```python
from build123d import *

# Parameters (mm, degrees)
BASE_PLATE_10MM_DEPTH         = 10
SUPPORT_BLOCK_50MM_DEPTH      = 25
SUPPORT_BLOCK_50MM_DEPTH_BACK = 25
ARCH_THROUGH_CUT_DEPTH        = 35
ARCH_THROUGH_CUT_DEPTH_BACK   = 35
UPPER_BOSS_SKETCH_W           = 20
UPPER_BOSS_SKETCH_H           = 10
UPPER_BOSS_3MM_DEPTH          = 3
BASE_PAD_SKETCH_W             = 20
BASE_PAD_SKETCH_H             = 10
BASE_PAD_4_19MM_DEPTH         = 4.19


with BuildPart() as part:
    # Base Plate Sketch → Base Plate 10mm (new body)
    with BuildSketch(Plane(origin=(0, 0, 0), x_dir=(1, 0, 0), z_dir=(0, 1, 0))):
        Polygon((60, 10), (42.8083356, 10), (42.8083356, -10), (60, -10), (60, -35), (-60, -35), (-60, -10), (-44.9850804, -10), (-44.9850804, 10), (-60, 10), (-60, 35), (60, 35), align=None)
    extrude(amount=BASE_PLATE_10MM_DEPTH)

    # Support Block Profile → Support Block 50mm (add, two sides: drawn at the far end of the back side and taken through both)
    with BuildSketch(Plane.XY.offset(-SUPPORT_BLOCK_50MM_DEPTH_BACK)):
        with BuildLine():
            Line((-40.889682702, 10), (-15, 10))
            ThreePointArc((-15, 10), (0, 25), (15, 10))
            Line((15, 10), (40.889682702, 10))
            Line((40.889682702, 10), (30, 49.749371855))
            Line((30, 49.749371855), (5, 49.749371855))
            Line((5, 49.749371855), (10, 41.089117817))
            Line((10, 41.089117817), (-10, 41.089117817))
            Line((-10, 41.089117817), (-5, 49.749371855))
            Line((-5, 49.749371855), (-30, 49.749371855))
            Line((-30, 49.749371855), (-40.889682702, 10))
        make_face()
        with BuildLine():
            ThreePointArc((15, 10), (0, 25), (-15, 10))
            Line((-15, 10), (0, 10))
            Line((0, 10), (15, 10))
        make_face()
    extrude(amount=SUPPORT_BLOCK_50MM_DEPTH + SUPPORT_BLOCK_50MM_DEPTH_BACK)

    # Arch Cut Sketch → Arch Through Cut (cut, two sides: drawn at the far end of the back side and taken through both)
    with BuildSketch(Plane.XY.offset(-ARCH_THROUGH_CUT_DEPTH_BACK)):
        with BuildLine():
            Line((-15, 10), (-15, 0))
            Line((-15, 0), (15, 0))
            Line((15, 0), (15, 10))
            ThreePointArc((15, 10), (0, 25), (-15, 10))
        make_face()
    extrude(amount=ARCH_THROUGH_CUT_DEPTH + ARCH_THROUGH_CUT_DEPTH_BACK, mode=Mode.SUBTRACT)

    # Upper Boss Sketch → Upper Boss 3mm (add)
    with BuildSketch(Plane(origin=(-44, 0, 0), x_dir=(0, 0, -1), z_dir=(1, 0, 0))):
        with Locations((0, 5)):
            Rectangle(UPPER_BOSS_SKETCH_W, UPPER_BOSS_SKETCH_H)
    extrude(amount=-UPPER_BOSS_3MM_DEPTH)

    # Base Pad Sketch → Base Pad 4.19mm (add)
    with BuildSketch(Plane(origin=(42.8083356, 0, 0), x_dir=(0, 0, -1), z_dir=(1, 0, 0))):
        with Locations((0, 5)):
            Rectangle(BASE_PAD_SKETCH_W, BASE_PAD_SKETCH_H)
    extrude(amount=BASE_PAD_4_19MM_DEPTH)


solid = part.part
```
Input: part model. Units: mm. Frame: model coordinates. A direction names the side the tool comes from. Give positions to 0.01 mm unless a question says otherwise; leave off trailing zeros. Order: outer loops, then holes, each group sorted by start corner. A loop starts at its lowest first (then second) coordinate and runs counter-clockwise, first axis right, second up. Notation, with made-up numbers: M 28,23 L 63,23 A23 cw 63,41 Z; hole C 58,-4.5 d9. An arc over 180 degrees is marked long. Return JSON: item names as keys, results as strings.
1) Section query A-A on x = -51.5. Output: boundary loops of the cut face in (y, z).
Taken from the geometry:
{"outline": "M 0,-35 L 10,-35 L 10,-10 L 0,-10 Z; M 0,10 L 10,10 L 10,35 L 0,35 Z"}
2) Access query for faces 4 (the face through (-15, 5, 0)), 5 (the face through (53, 5, 10)), 6 (the face through (-54, 5, 10)). Directions: +Z, -Z, +X, -X, +Y, -Y. A direction counts if a zero-diameter tool reaches every point of the face in a straight line with its end or side. Return the directions, or none.
Taken from the geometry:
{"face 4": "+Z, -Z, -Y", "face 5": "+X, +Y, -Y", "face 6": "-X, +Y, -Y"}
3) Section query C-C on y = 8. Output: boundary loops of the cut face in (x, z).
Taken from the geometry:
{"outline": "M -60,-35 L -15,-35 L -15,35 L -60,35 L -60,10 L -47,10 L -47,-10 L -60,-10 Z; M 15,-35 L 60,-35 L 60,-10 L 47,-10 L 47,10 L 60,10 L 60,35 L 15,35 Z"}
4) Section query B-B on z = -16. Output: boundary loops of the cut face in (x, y).
Taken from the geometry:
{"outline": "M -60,0 L -15,0 L -15,10 A15 cw 15,10 L 15,0 L 60,0 L 60,10 L 40.89,10 L 30,49.75 L 5,49.75 L 10,41.09 L -10,41.09 L -5,49.75 L -30,49.75 L -40.89,10 L -60,10 Z"}
5) Section query D-D on x = -26.5. Output: boundary loops of the cut face in (y, z).
Taken from the geometry:
{"outline": "M 0,-35 L 10,-35 L 10,-25 L 49.75,-25 L 49.75,25 L 10,25 L 10,35 L 0,35 Z"}
6) Contact query for flat-ended pins moving along their axis: pin 1 (1.5 mm diameter, centred on y = 39.5, z = -27, fed in from +X); pin 2 (5 mm diameter, centred on y = 22.5, z = 0.5, fed in from -X); pin 3 (3 mm diameter, centred on x = -7, y = 39.5, fed in from +Z); pin 4 (3 mm diameter, centred on y = 4, z = -3, fed in from -X). Output: stop coordinate, or through.
Taken from the geometry:
{"pin 1": "passes through", "pin 2": "stops at x = -38.15", "pin 3": "stops at z = 25", "pin 4": "stops at x = -47"}
7) Line query: L1, parallel to X at y = 9, z = 5.5; L2, parallel to X at y = 4.5, z = 25; L3, parallel to Z at x = 53, y = 8. Output: solid intervals per line, ascending. Write a range as [from, to].
Taken from the geometry:
{"L1": "x = [-47, -15], [15, 47]", "L2": "x = [-60, -15], [15, 60]", "L3": "z = [-35, -10], [10, 35]"}
8) Mould query, pull axis X, two halves, no side actions, for faces 1 (the face through (-60, 5, 23)), 2 (the face through (35.52, 29.6, -0.35)), 3 (the face through (-7.535, 45.359, -0.35)). Classes: released by +X, released by -X, zero draft, split by the parting line, or undercut.
Taken from the geometry:
{"face 1": "released by -X", "face 2": "released by +X", "face 3": "undercut"}
